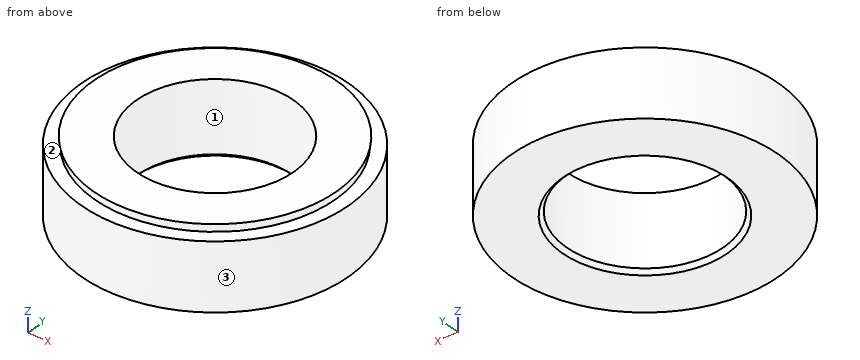
```python
from build123d import *

# Parameters (mm, degrees)
SKETCH_1_R          = 34
EXTRUDE_1_DEPTH     = 19
SKETCH_3_R          = 20
CUT_EXTRUDE_1_DEPTH = 52.701063819
CHAMFER_1_SIZE      = 1


with BuildPart() as part:
    # 草图1 → 凸台-拉伸1 (new body)
    with BuildSketch(Plane.XY):
        Circle(SKETCH_1_R)
    extrude(amount=EXTRUDE_1_DEPTH)

    # 草图2 → 切除-旋转1 (revolve, cut)
    with BuildSketch(Plane(origin=(0, 0, 0), x_dir=(1, 0, 0), z_dir=(0, 1, 0)), mode=Mode.PRIVATE) as cut_revolve_1_sk:
        with BuildLine():
            Line((-34, -17), (-30.626132632, -17))
            ThreePointArc((-30.626132632, -17), (-30.765967048, -17.997991107), (-30.873289426, -19))
            Line((-30.873289426, -19), (-34, -19))
            Line((-34, -19), (-34, -17))
        make_face()
    revolve(cut_revolve_1_sk.sketch.rotate(Axis((0, 0, 19), (0, 0, -1)), 180), axis=Axis((0, 0, 19), (0, 0, -1)), mode=Mode.SUBTRACT)

    # 草图3 → 切除-拉伸1 (cut, through all)
    with BuildSketch(Plane.XY.offset(19)):
        Circle(SKETCH_3_R)
    extrude(amount=-CUT_EXTRUDE_1_DEPTH, mode=Mode.SUBTRACT)

    # 倒角1
    chamfer_1_edges = [part.edges().sort_by_distance(p)[0] for p in [
        (-20, 0, 0),
    ]]
    chamfer(chamfer_1_edges, length=CHAMFER_1_SIZE)


solid = part.part
```
Work out the finished part from the listing and answer in its coordinate system (mm). Face numbers are marked on the shaded views. Give positions to 0.01 mm unless a question says otherwise; leave off trailing zeros. Order: outer loops, then holes, each group sorted by start corner. A loop starts at its lowest first (then second) coordinate and runs counter-clockwise, first axis right, second up. Notation, with made-up numbers: (62.5, 5.5) - (76.5, 5.5) arc R13 ccw to (76.5, 23.5) - close; hole circle Ø7 at (3.25, 40). An arc over 180 degrees is marked (long way). One line per item, written item: value. Start each with the question number.
1. Section A-A, the plane z = 10 is taken. Write down the section's boundary in (x, y).
2. For a pull along Y with two mould halves and no side action, classify the marked faces 1, 2 and 3 as released by +Y, released by -Y, zero draft, split by the parting line, or undercut.
3. Each of these flat-tipped pins is pushed along its axis until it touches: pin 1 Ø1.5 at (x, z) = (20.5, 8.5) entering from +Y; pin 2 Ø1 at (x, z) = (14.5, 13) entering from -Y; pin 3 Ø1 at (y, z) = (10, 5.5) entering from -X. Where does it stop, or does it pass through?
4. Consider line 1 (Y direction, x = 0, z = 15.5); line 2 (X direction, y = -0.5, z = 13.5); line 3 (Z direction, x = -7, y = 30.5). Determine where each line is inside the solid, lowest interval first.
Filled sheet:
1. outline: circle Ø68 at (0, 0); hole circle Ø40 at (0, 0)
2. face 1: undercut
2. face 2: zero draft
2. face 3: split by the parting line
3. pin 1: y = 27.68
3. pin 2: y = -30.98
3. pin 3: x = -32.65
4. line 1: -34 to -20, 20 to 34
4. line 2: -34 to -19.99, 19.99 to 34
4. line 3: 0 to 17
